Geometry: final body of the model. Coordinates: model frame, mm. Give positions to 0.01 mm unless a question says otherwise; leave off trailing zeros. Loops run counter-clockwise (first coordinate to the right, second up) from the corner with the lowest first, then second, coordinate; pieces in that order, holes last.
from build123d import *

# Parameters (mm, degrees)
SKETCH1_W           = 90
SKETCH1_H           = 12.5
BOSS_EXTRUDE1_DEPTH = 180
SKETCH2_W           = 66
SKETCH2_H           = 10
CUT_EXTRUDE1_DEPTH  = 186.960345235
CHAMFER1_SIZE       = 3
FILLET1_R           = 5
SKETCH3_W           = 15
SKETCH3_H           = 90
CUT_EXTRUDE2_DEPTH  = 186.960345235
SKETCH4_W           = 35
SKETCH4_H           = 120
CUT_EXTRUDE3_DEPTH  = 186.960345235
FILLET2_R           = 5
FILLET3_R           = 5


with BuildPart() as part:
    # Sketch1 → Boss-Extrude1 (new body)
    with BuildSketch(Plane.XY):
        Rectangle(SKETCH1_W, SKETCH1_H)
    extrude(amount=BOSS_EXTRUDE1_DEPTH)

    # Sketch2 → Cut-Extrude1 (cut, through all)
    with BuildSketch(Plane(origin=(0, 6.25, 0), x_dir=(1, 0, 0), z_dir=(0, 1, 0))):
        with Locations((0, -175)):
            Rectangle(SKETCH2_W, SKETCH2_H)
    extrude(amount=-CUT_EXTRUDE1_DEPTH, mode=Mode.SUBTRACT)

    # Chamfer1
    chamfer1_edges = [part.edges().sort_by_distance(p)[0] for p in [
        (39, 6.25, 180),
        (-39, 6.25, 180),
    ]]
    chamfer(chamfer1_edges, length=CHAMFER1_SIZE)

    # Fillet1
    fillet1_edges = [part.edges().sort_by_distance(p)[0] for p in [
        (39, 6.25, 177),
        (-39, 6.25, 177),
    ]]
    fillet(fillet1_edges, radius=FILLET1_R)

    # Sketch3 → Cut-Extrude2 (cut, through all)
    with BuildSketch(Plane(origin=(0, 6.25, 0), x_dir=(1, 0, 0), z_dir=(0, 1, 0))):
        with Locations((37.5, -45)):
            Rectangle(SKETCH3_W, SKETCH3_H)
        with Locations((-37.5, -45)):
            Rectangle(SKETCH3_W, SKETCH3_H)
    extrude(amount=-CUT_EXTRUDE2_DEPTH, mode=Mode.SUBTRACT)

    # Sketch4 → Cut-Extrude3 (cut, through all)
    with BuildSketch(Plane(origin=(0, 6.25, 0), x_dir=(1, 0, 0), z_dir=(0, 1, 0))):
        with Locations((0, -90)):
            Rectangle(SKETCH4_W, SKETCH4_H)
    extrude(amount=-CUT_EXTRUDE3_DEPTH, mode=Mode.SUBTRACT)

    # Fillet2
    fillet2_edges = [part.edges().sort_by_distance(p)[0] for p in [
        (-17.5, 0, 150),
        (-17.5, 0, 30),
        (17.5, 0, 30),
        (17.5, 0, 150),
    ]]
    fillet(fillet2_edges, radius=FILLET2_R)

    # Fillet3
    fillet3_edges = [part.edges().sort_by_distance(p)[0] for p in [
        (30, 0, 90),
        (-30, 0, 90),
    ]]
    fillet(fillet3_edges, radius=FILLET3_R)


solid = part.part
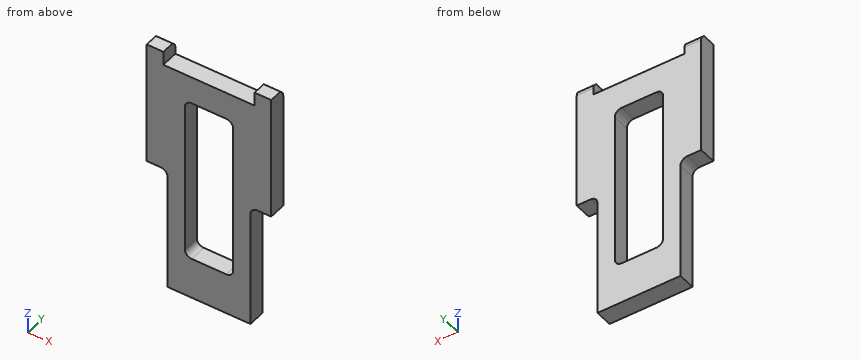
Item 1: Pin query (flat end, axial travel): pin 1 (2 mm diameter, centred on y = 5, z = 63.5, fed in from +X); pin 2 (5 mm diameter, centred on x = -42.5, y = 3, fed in from -Z); pin 3 (2 mm diameter, centred on x = 31, y = -0.5, fed in from +Z). Return the tip coordinate at first contact, or that it passes through.
Values follow:
pin 1: stops at x = 30
pin 2: stops at z = 90
pin 3: stops at z = 170
Item 2: Section query A-A on z = 123. Return loops of the section in (x, y), plus the area to 4 significant figures.
Values follow:
outline: (-45, -6.25) - (-17.5, -6.25) - (-17.5, 6.25) - (-45, 6.25) - close; (17.5, -6.25) - (45, -6.25) - (45, 6.25) - (17.5, 6.25) - close
area: 687.5 mm2
Item 3: Ray query, probe 1 along X at (y, z) = (-1, 139); probe 2 along X at (y, z) = (2, 36); probe 3 along Z at (x, y) = (14, 2). Return the intervals inside material, ascending.
Values follow:
probe 1: x = -45 to -17.5, 17.5 to 45
probe 2: x = -30 to -17.5, 17.5 to 30
probe 3: z = 0 to 30.23, 149.77 to 170
Item 4: Section query B-B on y = -1.5. Return loops of the section in (x, z).
Values follow:
outline: (-45, 90) - (-35, 90) arc R5 cw to (-30, 85) - (-30, 0) - (30, 0) - (30, 85) arc R5 cw to (35, 90) - (45, 90) - (45, 180) - (33, 180) - (33, 170) - (-33, 170) - (-33, 180) - (-45, 180) - close; hole (-17.5, 35) arc R5 ccw to (-12.5, 30) - (12.5, 30) arc R5 ccw to (17.5, 35) - (17.5, 145) arc R5 ccw to (12.5, 150) - (-12.5, 150) arc R5 ccw to (-17.5, 145) - close
Item 5: Section query D-D on x = 39. Return loops of the section in (y, z).
Values follow:
outline: (-6.25, 90) - (6.25, 90) - (6.25, 174.93) arc R5 ccw to (4.79, 178.46) - (3.25, 180) - (-6.25, 180) - close
Item 6: Section query C-C on x = 0. Return loops of the section in (y, z).
Values follow:
outline: (-6.25, 0) - (6.25, 0) - (6.25, 30) - (-6.25, 30) - close; (-6.25, 150) - (6.25, 150) - (6.25, 170) - (-6.25, 170) - close
